Source: three-view drawing plus pictorial views. Frame: mm from the lowest corner of the part. A direction names the side the tool comes from. Give positions to 0.01 mm unless a question says otherwise; leave off trailing zeros. Loops run counter-clockwise (first coordinate to the right, second up) from the corner with the lowest first, then second, coordinate; pieces in that order, holes last. Notation, with made-up numbers: (-31, -36) -> (-17, -36) arc R23 cw to (-17, -15) -> close; hole circle Ø3 at (42.5, -11). An arc over 180 degrees is marked (long way). One line per item, written item: value. Start each with the question number.
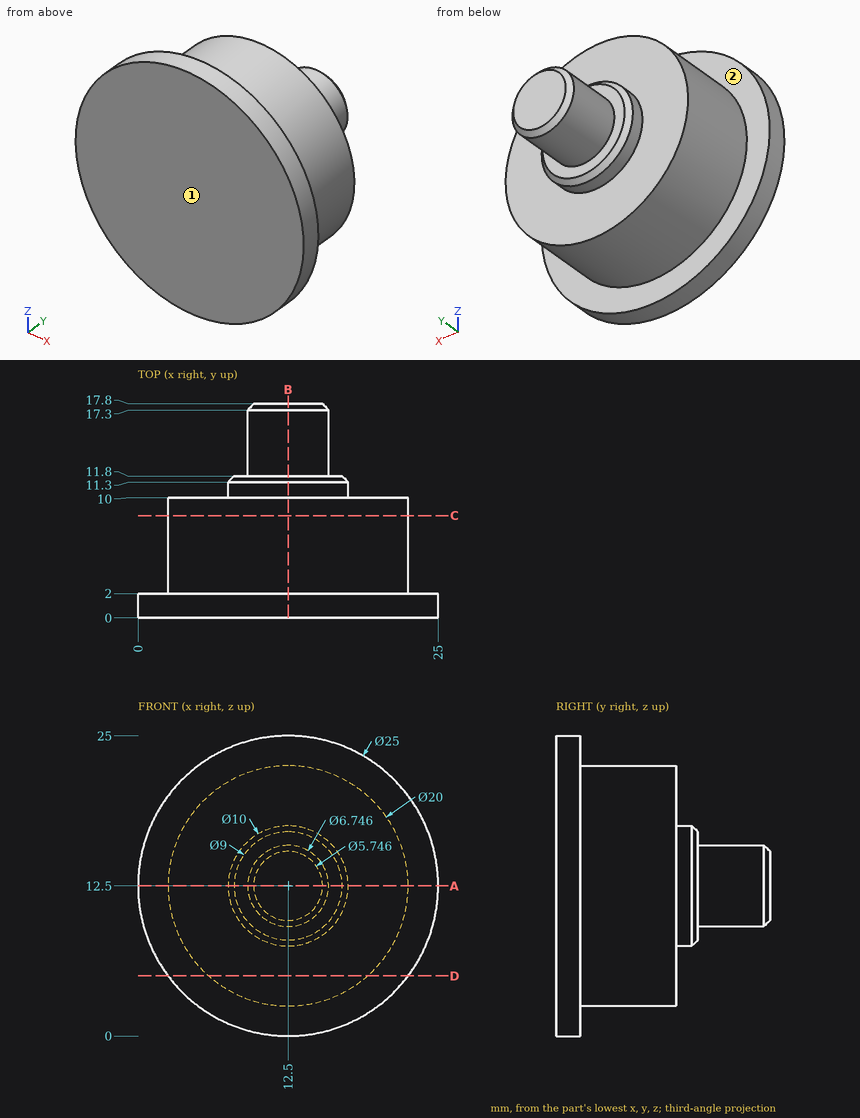
Item 1: Ray query, line 1 along Y through (x, z) = (15.5, 6.5); line 2 along Y through (x, z) = (3, 8.5); line 3 along X through (y, z) = (5.75, 12.5). Return the intervals inside material, ascending. Write a range as [from, to].
Item 2: Section D-D, the plane z = 5. Output: boundary loops of the cut face in (x, y) (1 decimal).
Item 3: Section C-C, the plane y = 8.5. Output: boundary loops of the cut face in (x, z).
Item 4: Access query for the marked faces 1 and 2. Directions: +Z, -Z, +X, -X, +Y, -Y. A direction counts if a zero-diameter tool reaches every point of the face in a straight line with its end or side. Return the directions, or none.
Item 5: Section B-B, the plane x = 12.5. Output: boundary loops of the cut face in (y, z).
Item 6: Pin query (flat end, axial travel): pin 1 (4 mm diameter, centred on x = 21, z = 9, fed in from +Y); pin 2 (6 mm diameter, centred on y = 10, z = 15, fed in from -X); pin 3 (3 mm diameter, centred on y = 7, z = 3.5, fed in from -X) (1 decimal). Return the tip coordinate at first contact, or that it passes through.
Item 7: Section A-A, the plane z = 12.5. Output: boundary loops of the cut face in (x, y), then the cut area to 3 significant figures.
Geometry check:
1. line 1: y = [0, 10]
1. line 2: y = [0, 2]
1. line 3: x = [2.5, 22.5]
2. outline: (2.5, 0) -> (22.5, 0) -> (22.5, 2) -> (19.1, 2) -> (19.1, 10) -> (5.9, 10) -> (5.9, 2) -> (2.5, 2) -> close
3. outline: circle Ø20 at (12.5, 12.5)
4. face 1: +Z, -Z, +X, -X, -Y
4. face 2: +Y
5. outline: (0, 0) -> (2, 0) -> (2, 2.5) -> (10, 2.5) -> (10, 7.5) -> (11.3, 7.5) -> (11.8, 8) -> (11.8, 9.13) -> (17.3, 9.13) -> (17.8, 9.63) -> (17.8, 15.37) -> (17.3, 15.87) -> (11.8, 15.87) -> (11.8, 17) -> (11.3, 17.5) -> (10, 17.5) -> (10, 22.5) -> (2, 22.5) -> (2, 25) -> (0, 25) -> close
6. pin 1: stops at y = 10
6. pin 2: stops at x = 2.5
6. pin 3: stops at x = 5.9
7. outline: (0, 0) -> (25, 0) -> (25, 2) -> (22.5, 2) -> (22.5, 10) -> (17.5, 10) -> (17.5, 11.3) -> (17, 11.8) -> (15.87, 11.8) -> (15.87, 17.3) -> (15.37, 17.8) -> (9.63, 17.8) -> (9.13, 17.3) -> (9.13, 11.8) -> (8, 11.8) -> (7.5, 11.3) -> (7.5, 10) -> (2.5, 10) -> (2.5, 2) -> (0, 2) -> close
7. area: 268 mm2
